from build123d import *

# Parameters (mm, degrees)
SKETCH1_R           = 50
BOSS_EXTRUDE1_DEPTH = 138
BOSS_EXTRUDE2_START = -14
SKETCH6_R           = 71
SKETCH6_R_2         = 50
BOSS_EXTRUDE2_DEPTH = 14
CHAMFER3_SIZE       = 1
CHAMFER4_SIZE       = 1
CHAMFER5_SIZE       = 1
SKETCH7_R           = 17.5
CUT_EXTRUDE1_DEPTH  = 7
CHAMFER6_SIZE       = 1
CIRPATTERN1_COUNT   = 6
M8_TAPPED_HOLE1_D   = 6.8


with BuildPart() as part:
    # Sketch1 → Boss-Extrude1 (new body)
    with BuildSketch(Plane.XY):
        Circle(SKETCH1_R)
    extrude(amount=BOSS_EXTRUDE1_DEPTH)

    # Sketch6 → Boss-Extrude2 (add)
    with BuildSketch(Plane.XY.offset(138).offset(BOSS_EXTRUDE2_START)):
        Circle(SKETCH6_R)
        Circle(SKETCH6_R_2, mode=Mode.SUBTRACT)
    extrude(amount=BOSS_EXTRUDE2_DEPTH)

    # Chamfer3
    chamfer3_edges = [part.edges().sort_by_distance(p)[0] for p in [
        (-50, 0, 0),
    ]]
    chamfer(chamfer3_edges, length=CHAMFER3_SIZE)

    # Chamfer4
    chamfer4_edges = [part.edges().sort_by_distance(p)[0] for p in [
        (-71, 0, 138),
    ]]
    chamfer(chamfer4_edges, length=CHAMFER4_SIZE)

    # Chamfer5
    chamfer5_edges = [part.edges().sort_by_distance(p)[0] for p in [
        (-71, 0, 124),
    ]]
    chamfer(chamfer5_edges, length=CHAMFER5_SIZE)

    # Sketch7 → Cut-Extrude1 (cut)
    with BuildSketch(Plane.XY.offset(138)):
        Circle(SKETCH7_R)
    extrude(amount=-CUT_EXTRUDE1_DEPTH, mode=Mode.SUBTRACT)

    # Chamfer6
    chamfer6_edges = [part.edges().sort_by_distance(p)[0] for p in [
        (-17.5, 0, 138),
    ]]
    chamfer(chamfer6_edges, length=CHAMFER6_SIZE)

    # Sketch9 → Hole size (per socket head cap screw type)1 (revolve, cut)
    with BuildSketch(Plane(origin=(60, 0, 138), x_dir=(0, -1, 0), z_dir=(1, 0, 0))):
        Polygon((0, 0), (0, 15.652366702), (2.75, 14), (2.75, 7), (5, 7), (5, 0), align=None)
    hole_size_per_socket_head_cap_screw_typ = revolve(axis=Axis((60, 0, 144.35), (0, 0, -1)), mode=Mode.SUBTRACT)

    # CirPattern1: Hole size (per socket head cap screw type)1 ×6 about axis
    cirpattern1_axis = Axis((0, 0, 0), (0, 0, 1))
    for i in range(1, CIRPATTERN1_COUNT):
        add(hole_size_per_socket_head_cap_screw_typ.rotate(cirpattern1_axis, i * 360 / CIRPATTERN1_COUNT), mode=Mode.SUBTRACT)

    # M8 Tapped Hole1 (through all)
    with Locations(Plane.XY.offset(138)):
        with Locations((0, 61), (0, -61)):
            Hole(M8_TAPPED_HOLE1_D / 2)


solid = part.part
Geometry check sheet. Reference: the model listing, model coordinates, mm. A direction names the side the tool comes from. Round coordinates to 2 decimals unless told otherwise and drop trailing zeros. Order: outer loops, then holes, each group sorted by start corner. A loop starts at its lowest first (then second) coordinate and runs counter-clockwise, first axis right, second up. Notation, with made-up numbers: (-24.5, 23) - (-20.5, 23) arc R17 cw to (-20.5, 28) - close; hole circle Ø6 at (18.25, 1.25). An arc over 180 degrees is marked (long way). One line per question, with ' | ' between items. Start each with the question number.
(1) Release check for a two-part mould opening along X. For faces 1 (the cylindrical face through (-15.39, -69.31, 130.92)), 2 (the cylindrical face through (-34.216, 49.274, 134.549)), 3 (the flat face through (15, -15, 138)) record: released by +X, released by -X, zero draft, split by the parting line, or undercut.
(2) Sectioned sample at A-A on x = 0. Record the cut outline in (y, z), and give its area (3 significant figures).
(3) Depth check by flat-ended pin: pin 1 Ø6 at (x, y) = (30, 51.96) entering from +Z; pin 2 Ø8 at (y, z) = (-41, 107) entering from +X; pin 3 Ø11 at (x, y) = (0, 61) entering from +Z; pin 4 Ø2 at (x, z) = (2, 82.5) entering from -Y. Enter the tip coordinate at first touch or a pass-through.
(4) Sectioned sample at C-C on z = 65. Record the cut outline in (x, y), and give its area (3 significant figures).
(5) Sectioned sample at B-B on y = 0. Count the separate pieces of the cut face and the enclosed holes in it, and give its area (3 significant figures).
(6) Access from +Z, -Z, +X, -X, +Y, -Y to the whole of each face (thin tool, end or side, straight path). Record for faces 4 (the cylindrical face through (-28.947, -54.502, 127.549)), 5 (the cylindrical face through (-55.043, -0.651, 134.549)).
(7) Thickness scan on L1, parallel to Y at x = 0, z = 133.25; L2, parallel to Z at x = -41.5, y = 35; L3, parallel to Z at x = -4.5, y = -15. Record the ranges inside material, lowest first. Write a range as [from, to].
Conclusion:
1) face 1: split by the parting line | face 2: undercut | face 3: zero draft
2) outline: (-71, 125) - (-70, 124) - (-64.4, 124) - (-64.4, 138) - (-70, 138) - (-71, 137) - close; (-57.6, 124) - (-50, 124) - (-50, 1) - (-49, 0) - (49, 0) - (50, 1) - (50, 124) - (57.6, 124) - (57.6, 138) - (18.5, 138) - (17.5, 137) - (17.5, 131) - (-17.5, 131) - (-17.5, 137) - (-18.5, 138) - (-57.6, 138) - close; (64.4, 124) - (70, 124) - (71, 125) - (71, 137) - (70, 138) - (64.4, 138) - close | area: 13,900 mm2
3) pin 1: stops at z = 131 | pin 2: stops at x = 33.63 | pin 3: stops at z = 138 | pin 4: stops at y = -49.99
4) outline: circle Ø100 at (0, 0) | area: 7,850 mm2
5) separate pieces: 3 | enclosed holes: 0 | area: 13,900 mm2
6) face 4: +Z, -Z | face 5: +Z
7) L1: y = [-71, -64.4], [-57.6, -17.5], [17.5, 57.6], [64.4, 71] | L2: z = [124, 138] | L3: z = [0, 131]
